Could you check a few things on this model? Use its own coordinates, in mm. A direction names the side the tool comes from. Give positions to 0.01 mm unless a question says otherwise; leave off trailing zeros. Order: outer loops, then holes, each group sorted by start corner. A loop starts at its lowest first (then second) coordinate and runs counter-clockwise, first axis right, second up. Notation, with made-up numbers: (-13.5, 23) -> (1.5, 23) arc R15 cw to (1.5, 31) -> close; hole circle Ø9 at (63.25, 26.5). An arc over 180 degrees is marked (long way). One line per item, written item: value.
```python
from build123d import *

# Parameters (mm, degrees)
SKETCH_1_W             = 196.5
SKETCH_1_H             = 217
SKETCH_1_R             = 74
EXTRUDE_1_DEPTH        = 12
SKETCH_2_R             = 91.25
CUT_EXTRUDE_1_DEPTH    = 2
CUT_EXTRUDE_START      = -2
SKETCH_3_R             = 91.25
CUT_EXTRUDE_2_DEPTH    = 2
HOLE_WIZARD_M6_1_D     = 6.6
HOLE_WIZARD_M8_1_D     = 6.8
HOLE_WIZARD_M8_1_DEPTH = 19.75
HOLE_WIZARD_M8_1_TIP   = 2.042926105
HOLE_WIZARD_M8_2_D     = 6.8
HOLE_WIZARD_M8_2_DEPTH = 19.75
HOLE_WIZARD_M8_2_TIP   = 2.042926105


with BuildPart() as part:
    # 草图1 → 凸台-拉伸1 (new body)
    with BuildSketch(Plane.XY):
        Rectangle(SKETCH_1_W, SKETCH_1_H)
        Circle(SKETCH_1_R, mode=Mode.SUBTRACT)
    extrude(amount=EXTRUDE_1_DEPTH)

    # 草图2 → 切除-拉伸1 (cut)
    with BuildSketch(Plane(origin=(0, 0, 0), x_dir=(-1, 0, 0), z_dir=(0, 0, -1))):
        Circle(SKETCH_2_R)
    extrude(amount=-CUT_EXTRUDE_1_DEPTH, mode=Mode.SUBTRACT)

    # 草图3 → 切除-拉伸2 (cut)
    with BuildSketch(Plane.XY.offset(12).offset(CUT_EXTRUDE_START)):
        with Locations(Location((0, 0, 0), (0, 0, 180))):
            Circle(SKETCH_3_R)
    extrude(amount=CUT_EXTRUDE_2_DEPTH, mode=Mode.SUBTRACT)

    # M6 间隙孔1 (through all)
    with Locations(Plane.XY.offset(10)):
        with Locations((0, 84), (42, 72.746133918), (72.746133918, 42), (84, 0), (72.746133918, -42), (42, -72.746133918), (0, -84), (-42, -72.746133918), (-72.746133918, -42), (-84, 0), (-72.746133918, 42), (-42, 72.746133918)):
            Hole(HOLE_WIZARD_M6_1_D / 2)

    # M8 螺纹孔1
    with Locations(Plane.ZY.offset(98.25)):
        with Locations((6, 95), (6, 40), (6, -40), (6, -95)):
            Hole(HOLE_WIZARD_M8_1_D / 2, depth=HOLE_WIZARD_M8_1_DEPTH)
            with Locations((0, 0, -(HOLE_WIZARD_M8_1_DEPTH + HOLE_WIZARD_M8_1_TIP / 2))):  # 118° drill point
                Cone(0, HOLE_WIZARD_M8_1_D / 2, HOLE_WIZARD_M8_1_TIP, mode=Mode.SUBTRACT)

    # M8 螺纹孔2
    with Locations(Plane(origin=(98.25, 0, 0), x_dir=(0, 0, -1), z_dir=(1, 0, 0))):
        with Locations((-6, 95), (-6, 40), (-6, -40), (-6, -95)):
            Hole(HOLE_WIZARD_M8_2_D / 2, depth=HOLE_WIZARD_M8_2_DEPTH)
            with Locations((0, 0, -(HOLE_WIZARD_M8_2_DEPTH + HOLE_WIZARD_M8_2_TIP / 2))):  # 118° drill point
                Cone(0, HOLE_WIZARD_M8_2_D / 2, HOLE_WIZARD_M8_2_TIP, mode=Mode.SUBTRACT)


solid = part.part
```
1) Suppose I cut it at C-C, the plane x = -64. Write out the boundary of the cut face in (y, z), then the cut area to 3 significant figures.
Answer below:
outline: (-108.5, 0) -> (-65.04, 0) -> (-65.04, 2) -> (-37.15, 2) -> (-37.15, 10) -> (-65.04, 10) -> (-65.04, 12) -> (-108.5, 12) -> close; (37.15, 2) -> (65.04, 2) -> (65.04, 0) -> (108.5, 0) -> (108.5, 12) -> (65.04, 12) -> (65.04, 10) -> (37.15, 10) -> close
area: 1,490 mm2
2) We'd pull the mould along X, two halves only. Please class faces 5 (the flat face through (-1, 108.5, 6)), 6 (the conical face through (-76.812, -40.576, 5.872)), 7 (the cylindrical face through (76.043, 42.145, 5.944)), 8 (the flat face through (-6, 74, 10)): +X half, -X half, draft (parallel to the pull), parting line (faces both ways), or undercut.
Answer below:
face 5: draft
face 6: -X half
face 7: undercut
face 8: undercut
3) If I drill on line 1 along Y through (x, z) = (84, 5.5); line 2 along Y through (x, z) = (41.5, 6.25); line 3 along Z through (x, y) = (92.75, 95), over which ranges is the centre line in solid material (lowest first)?
Answer below:
line 1: y = -108.5 to -98.36, -91.64 to -43.36, -36.64 to -3.3, 3.3 to 36.64, 43.36 to 91.64, 98.36 to 108.5
line 2: y = -108.5 to -76.01, -69.48 to -61.27, 61.27 to 69.48, 76.01 to 108.5
line 3: z = 0 to 2.6, 9.4 to 12
4) Suppose I cut it at D-D, the plane x = -84. Write out the boundary of the cut face in (y, z), then the cut area to 3 significant figures.
Answer below:
outline: (-108.5, 0) -> (-35.64, 0) -> (-35.64, 2) -> (-3.3, 2) -> (-3.3, 10) -> (-35.64, 10) -> (-35.64, 12) -> (-108.5, 12) -> close; (3.3, 2) -> (35.64, 2) -> (35.64, 0) -> (108.5, 0) -> (108.5, 12) -> (35.64, 12) -> (35.64, 10) -> (3.3, 10) -> close; hole circle Ø6.8 at (-95, 6); hole circle Ø6.8 at (-40, 6); hole circle Ø6.8 at (40, 6); hole circle Ø6.8 at (95, 6)
area: 2,120 mm2
5) Suppose I cut it at A-A, the plane x = 0. Write out the boundary of the cut face in (y, z).
Answer below:
outline: (-108.5, 0) -> (-91.25, 0) -> (-91.25, 2) -> (-87.3, 2) -> (-87.3, 10) -> (-91.25, 10) -> (-91.25, 12) -> (-108.5, 12) -> close; (-80.7, 2) -> (-74, 2) -> (-74, 10) -> (-80.7, 10) -> close; (74, 2) -> (80.7, 2) -> (80.7, 10) -> (74, 10) -> close; (87.3, 2) -> (91.25, 2) -> (91.25, 0) -> (108.5, 0) -> (108.5, 12) -> (91.25, 12) -> (91.25, 10) -> (87.3, 10) -> close
6) For faces 1 (the cylindrical face through (88.2, 92, 7.6)), 2 (the cylindrical face through (-1.774, -81.217, 5.944)), 3 (the flat face through (-6, -74, 2)), 4 (the cylindrical face through (-88.2, 92, 4.4)), which set-ups out of +Z, -Z, +X, -X, +Y, -Y let a thin tool reach every point of the face, with its end or its side?
Answer below:
face 1: +X
face 2: +Z, -Z
face 3: -Z
face 4: -X
7) Suppose I cut it at B-B, the plane y = -53.5. Write out the boundary of the cut face in (x, z).
Answer below:
outline: (-98.25, 0) -> (-73.92, 0) -> (-73.92, 2) -> (-51.12, 2) -> (-51.12, 10) -> (-73.92, 10) -> (-73.92, 12) -> (-98.25, 12) -> close; (51.12, 2) -> (73.92, 2) -> (73.92, 0) -> (98.25, 0) -> (98.25, 12) -> (73.92, 12) -> (73.92, 10) -> (51.12, 10) -> close
8) For P1, Ø7.5, axis at x = 42, y = 72.75, coming from the -Z side; P2, Ø6, axis at x = 36, y = -63, coming from the +Z side; P3, Ø4, axis at y = -40, z = 6, coming from the -X side, each with a flat end and sliding along its axis, tell me the tip position at first contact or that it passes through.
Answer below:
P1: stops at z = 2
P2: stops at z = 10
P3: stops at x = -77.66
